```python
from build123d import *

# Parameters (mm, degrees)
SKETCH1_W           = 120
SKETCH1_H           = 90
BOSS_EXTRUDE1_DEPTH = 10
SKETCH2_R           = 7.5
CUT_EXTRUDE1_DEPTH  = 10
CHAMFER1_SIZE       = 5


with BuildPart() as part:
    # Sketch1 → Boss-Extrude1 (new body)
    with BuildSketch(Plane.XY):
        Rectangle(SKETCH1_W, SKETCH1_H)
    extrude(amount=BOSS_EXTRUDE1_DEPTH)

    # Sketch2 → Cut-Extrude1 (cut)
    with BuildSketch(Plane.XY.offset(10)):
        with Locations((-40, 30)):
            Circle(SKETCH2_R)
    extrude(amount=-CUT_EXTRUDE1_DEPTH, mode=Mode.SUBTRACT)

    # Chamfer1
    chamfer1_edges = [part.edges().sort_by_distance(p)[0] for p in [
        (-60, 45, 5),
        (60, 45, 5),
    ]]
    chamfer(chamfer1_edges, length=CHAMFER1_SIZE)


solid = part.part
```
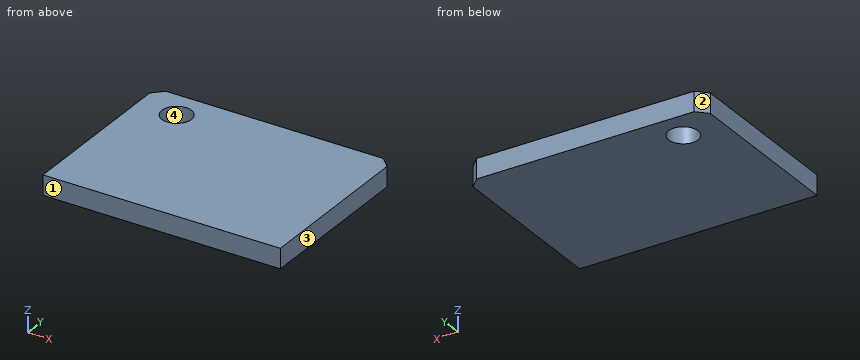
Check sheet for the modelled part. Datum: model origin and axes. Units: mm. Face numbers are marked on the shaded views. Give positions to 0.01 mm unless a question says otherwise; leave off trailing zeros. Write each loop counter-clockwise with the first axis right and the second up, starting at its lowest first coordinate (ties: lowest second). Pieces come first, ordered by that corner, then holes.
Item 1: Cross-section at B-B (z = 4.25). Enter the section's corners in (x, y), and give its area (3 significant figures).
Item 2: Cross-section at A-A (x = -40). Enter the section's corners in (y, z).
Item 3: Draft check along Y on the marked faces 1, 2, 3 and 4. Enter one of: released by +Y, released by -Y, zero draft, split by the parting line, or undercut.
Item 4: Cross-section at C-C (y = 30). Enter the section's corners in (x, z), and give its area (3 significant figures).
Item 5: Scan line: L1, parallel to Y at x = -40, z = 6.5. Record every from-to range of solid material in increasing order.
Report:
1. outline: (-60, -45) - (60, -45) - (60, 40) - (55, 45) - (-55, 45) - (-60, 40) - close; hole circle Ø15 at (-40, 30)
1. area: 10,600 mm2
2. outline: (-45, 0) - (22.5, 0) - (22.5, 10) - (-45, 10) - close; (37.5, 0) - (45, 0) - (45, 10) - (37.5, 10) - close
3. face 1: released by -Y
3. face 2: released by +Y
3. face 3: zero draft
3. face 4: undercut
4. outline: (-60, 0) - (-47.5, 0) - (-47.5, 10) - (-60, 10) - close; (-32.5, 0) - (60, 0) - (60, 10) - (-32.5, 10) - close
4. area: 1,050 mm2
5. L1: y = -45 to 22.5, 37.5 to 45
